The listing builds one solid part. Answer for the finished solid, in the listing's coordinates (mm). Face numbers are marked on the shaded views. Give positions to 0.01 mm unless a question says otherwise; leave off trailing zeros. Write each loop counter-clockwise with the first axis right and the second up, starting at its lowest first coordinate (ties: lowest second). Pieces come first, ordered by that corner, then holes. Notation, with made-up numbers: (27, 62.25) -> (74, 62.25) arc R27 cw to (74, 80.25) -> close; hole circle Ø3 at (61, 26). An arc over 180 degrees is marked (long way). One line per question, with ' | ' between items.
from build123d import *

# Parameters (mm, degrees)
SKETCH1_R          = 4.188125
BOSS_EXTRUDE_DEPTH = 9.5
SKETCH2_OUTSIDE_W  = 80.144
SKETCH2_OUTSIDE_H  = 77.786
SKETCH2_OUTSIDE_R  = 7.621023553
CUT_EXTRUDE1_DEPTH = 16.025644745
CUT_EXTRUDE1_DRAFT = -60
SKETCH3_OUTSIDE_W  = 80.144
SKETCH3_OUTSIDE_H  = 77.786
SKETCH3_OUTSIDE_R  = 7.621023553
CUT_EXTRUDE2_DEPTH = 16.025644745
CUT_EXTRUDE2_DRAFT = -60
CHAMFER1_SIZE      = 0.2375


with BuildPart() as part:
    # Sketch1 → Boss-Extrude (new body)
    with BuildSketch(Plane.XY):
        Polygon((4.4, 7.621023553), (-4.4, 7.621023553), (-8.8, 0), (-4.4, -7.621023553), (4.4, -7.621023553), (8.8, 0), align=None)
        Circle(SKETCH1_R, mode=Mode.SUBTRACT)
    extrude(amount=BOSS_EXTRUDE_DEPTH)


with BuildPart() as cut_extrude1_tool:
    # Sketch2 outside → Cut-Extrude1 (with draft: the straight prism first)
    with BuildSketch(Plane(origin=(0, 0, 0), x_dir=(-1, 0, 0), z_dir=(0, 0, -1))):
        Rectangle(SKETCH2_OUTSIDE_W, SKETCH2_OUTSIDE_H)
        Circle(SKETCH2_OUTSIDE_R, mode=Mode.SUBTRACT)
    extrude(amount=-CUT_EXTRUDE1_DEPTH)
    # Cut-Extrude1: the draft: its side faces are tilted about the plane it starts from
    cut_extrude1_sides = [cut_extrude1_tool.faces().sort_by_distance(p)[0] for p in [
        (0, -38.893, 8.012822372),
        (-40.072, 0, 8.012822372),
        (0, 38.893, 8.012822372),
        (40.072, 0, 8.012822372),
        (7.621023553, 0, 8.012822372),
    ]]
    draft(cut_extrude1_sides, Plane(origin=(0, 0, 0), x_dir=(-1, 0, 0), z_dir=(0, 0, -1)), CUT_EXTRUDE1_DRAFT)


with BuildPart() as part_1:
    add(part.part)

    # Cut-Extrude1: cut by cut_extrude1_tool
    add(cut_extrude1_tool.part, mode=Mode.SUBTRACT)


with BuildPart() as cut_extrude2_tool:
    # Sketch3 outside → Cut-Extrude2 (with draft: the straight prism first)
    with BuildSketch(Plane.XY.offset(9.5)):
        Rectangle(SKETCH3_OUTSIDE_W, SKETCH3_OUTSIDE_H)
        Circle(SKETCH3_OUTSIDE_R, mode=Mode.SUBTRACT)
    extrude(amount=-CUT_EXTRUDE2_DEPTH)
    # Cut-Extrude2: the draft: its side faces are tilted about the plane it starts from
    cut_extrude2_sides = [cut_extrude2_tool.faces().sort_by_distance(p)[0] for p in [
        (0, -38.893, 1.487177628),
        (40.072, 0, 1.487177628),
        (0, 38.893, 1.487177628),
        (-40.072, 0, 1.487177628),
        (-7.621023553, 0, 1.487177628),
    ]]
    draft(cut_extrude2_sides, Plane.XY.offset(9.5), CUT_EXTRUDE2_DRAFT)


with BuildPart() as part_2:
    add(part_1.part)

    # Cut-Extrude2: cut by cut_extrude2_tool
    add(cut_extrude2_tool.part, mode=Mode.SUBTRACT)

    # Chamfer1
    chamfer1_edges = [part_2.edges().sort_by_distance(p)[0] for p in [
        (-4.188125, 0, 0),
        (-4.188125, 0, 9.5),
    ]]
    chamfer(chamfer1_edges, length=CHAMFER1_SIZE)


solid = part_2.part
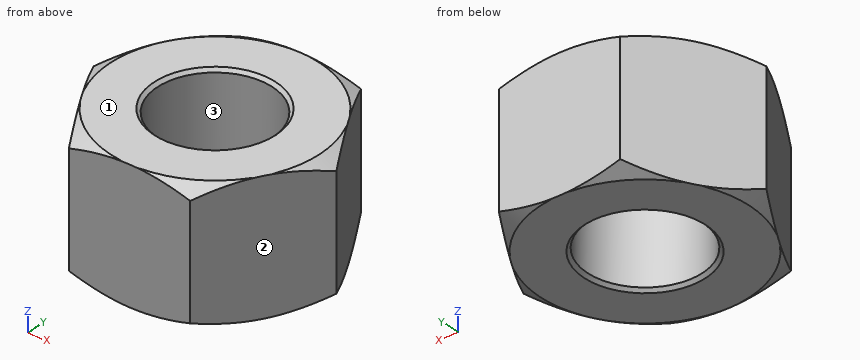
Item 1: Determine the mould class of the marked faces 1, 2 and 3 for opening direction X: pulls with the +X half, pulls with the -X half, needs draft (parallel to the pull), parting line crosses it, or undercut.
Answers below:
face 1: needs draft | face 2: pulls with the +X half | face 3: undercut
Item 2: Flat-ended cylindrical pins translate along their axes: pin 1 (1.5 mm diameter, centred on y = 2, z = 7, fed in from -X); pin 2 (2 mm diameter, centred on y = -4.5, z = 7.5, fed in from -X). Find the tip coordinate at first contact, or state that the pin passes through.
Answers below:
pin 1: x = -8.08 | pin 2: x = -6.78
Item 3: Consider line 1 (Y direction, x = 0, z = 3); line 2 (Y direction, x = 1.75, z = 4); line 3 (X direction, y = -5.75, z = 6.5). Determine where each line is inside the solid, lowest interval first. Write a range as [from, to].
Answers below:
line 1: [-7.62, -4.19], [4.19, 7.62] | line 2: [-7.62, -3.8], [3.8, 7.62] | line 3: [-5.48, 5.48]
Item 4: Find section A-A (z = 3.75). Write down the section's boundary in (x, y).
Answers below:
outline: (-8.8, 0) -> (-4.4, -7.62) -> (4.4, -7.62) -> (8.8, 0) -> (4.4, 7.62) -> (-4.4, 7.62) -> close; hole circle Ø8.38 at (0, 0)
